For this review, use the dimensioned drawing (mm, ordinates from the lowest corner) and the shaded views. A direction names the side the tool comes from. Give positions to 0.01 mm unless a question says otherwise; leave off trailing zeros. Write each loop counter-clockwise with the first axis right and the second up, starting at its lowest first coordinate (ties: lowest second). Pieces come first, ordered by that corner, then holes. Notation, with made-up numbers: M -3,10 L 33,10 A21 ccw 33,14 Z; hole C -21.75,-35 d4. An arc over 180 degrees is marked long. Answer in a Markdown table with one row per item.
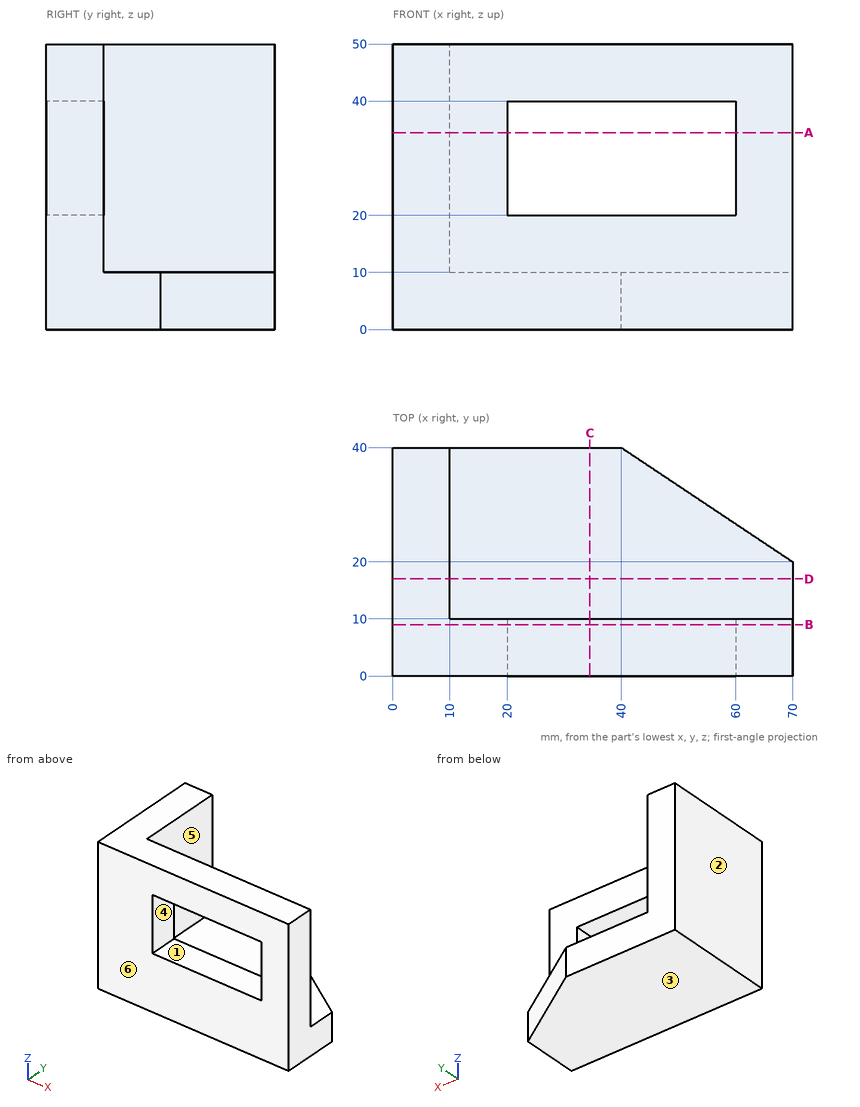
1) Add section B-B (y = 9). Write out the cut boundary in (x, z).
Geometry says:
| item | result |
|---|---|
| outline | M 0,0 L 70,0 L 70,50 L 0,50 Z; hole M 20,20 L 60,20 L 60,40 L 20,40 Z |
2) Add section A-A (z = 34.5). Write out the cut boundary in (x, y), and give its area (3 significant figures).
Geometry says:
| item | result |
|---|---|
| outline | M 0,0 L 20,0 L 20,10 L 10,10 L 10,40 L 0,40 Z; M 60,0 L 70,0 L 70,10 L 60,10 Z |
| area | 600 mm^2 |
3) Add section D-D (y = 17). Write out the cut boundary in (x, z).
Geometry says:
| item | result |
|---|---|
| outline | M 0,0 L 70,0 L 70,10 L 10,10 L 10,50 L 0,50 Z |
4) The part is to be moulded in two halves that separate along Z. For the marked faces 1, 2 and 3, say which applies: released by +Z, released by -Z, zero draft, split by the parting line, or undercut.
Geometry says:
| item | result |
|---|---|
| face 1 | undercut |
| face 2 | zero draft |
| face 3 | released by -Z |
5) To check wall thickness, follow probe 1 along X at (y, z) = (6.5, 35); probe 2 along Y at (x, z) = (11.5, 28.5); probe 3 along Z at (x, y) = (36.5, 3). State the ranges of each line that lie inside material, in increasing order. Write a range as [from, to].
Geometry says:
| item | result |
|---|---|
| probe 1 | [0, 20], [60, 70] |
| probe 2 | [0, 10] |
| probe 3 | [0, 20], [40, 50] |
6) Insertion check: P1, Ø9, axis at y = 28.5, z = 35.5, coming from the +X side; P2, Ø5, axis at y = 15.5, z = 45, coming from the -X side; P3, Ø20, axis at x = 29.5, z = 22, coming from the +Y side; P4, Ø1, axis at x = 42.5, y = 13.5, coming from the +Z side. Each pin has a flat end and moves straight along its axis. Give the tip position at first contact, or say it passes through.
Geometry says:
| item | result |
|---|---|
| P1 | x = 10 |
| P2 | x = 0 |
| P3 | y = 10 |
| P4 | z = 10 |
7) For the marked faces 4, 5 and 6, list the 3-axis set-ups (+Z, -Z, +X, -X, +Y, -Y) from which the entire face can be reached by the end or side of a thin tool; tool diameter is ignored.
Geometry says:
| item | result |
|---|---|
| face 4 | +Y, -Y |
| face 5 | +Z, +X, +Y |
| face 6 | +Z, -Z, +X, -X, -Y |
8) Add section C-C (x = 34.5). Write out the cut boundary in (y, z), and give its area (3 significant figures).
Geometry says:
| item | result |
|---|---|
| outline | M 0,0 L 40,0 L 40,10 L 10,10 L 10,20 L 0,20 Z; M 0,40 L 10,40 L 10,50 L 0,50 Z |
| area | 600 mm^2 |
